Print and shaded views of the part. All mm, measured from the part's lowest x, y and z. Round coordinates to 2 decimals unless told otherwise and drop trailing zeros. Write each loop counter-clockwise with the first axis right and the second up, starting at its lowest first coordinate (ties: lowest second). Pieces come first, ordered by that corner, then holes. Notation, with made-up numbers: M 9.25,15 L 63.25,15 A24 ccw 63.25,48 Z; hole C -28.75,65.25 d3. An arc over 180 degrees is marked long. Write item = value, one per line.
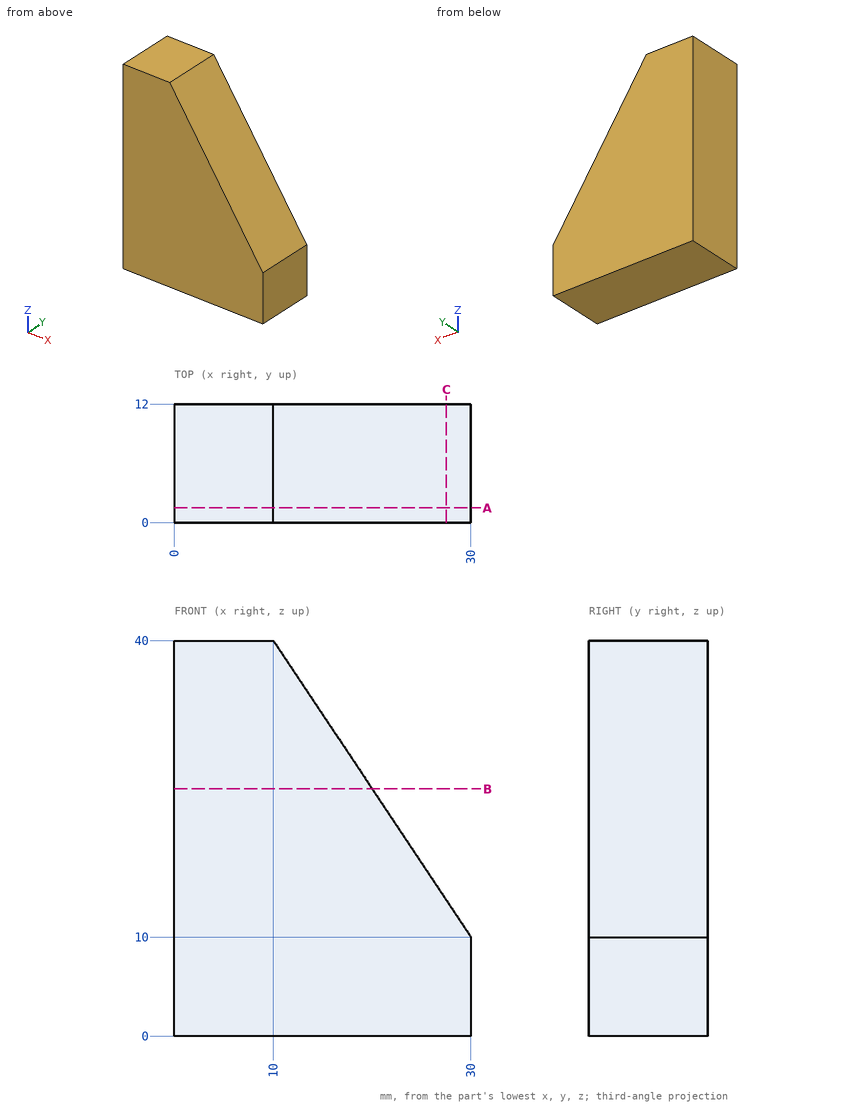
1. Band-saw the part on A-A (y = 1.5). List the corners of the cut face in (x, z).
Responses:
outline = M 0,0 L 30,0 L 30,10 L 10,40 L 0,40 Z
2. Band-saw the part on C-C (x = 27.5). List the corners of the cut face in (y, z), plus the area to 3 significant figures.
Responses:
outline = M 0,0 L 12,0 L 12,13.75 L 0,13.75 Z
area = 165 mm²
3. Band-saw the part on B-B (z = 25). List the corners of the cut face in (x, y), plus the area to 3 significant figures.
Responses:
outline = M 0,0 L 20,0 L 20,12 L 0,12 Z
area = 240 mm²
4. Probe probe 1 along X at (y, z) = (1.75, 37); probe 2 along X at (y, z) = (2, 24); probe 3 along Z at (x, y) = (22.75, 7.5) (3 decimals). List the from-to ranges inside material, lowest first.
Responses:
probe_1 = 0 to 12
probe_2 = 0 to 20.67
probe_3 = 0 to 20.875
